Job drawing, mm, ordinate dimensions from the low corner. One solid piece. A direction names the side the tool comes from. Round coordinates to 2 decimals unless told otherwise and drop trailing zeros. Write each loop counter-clockwise with the first axis right and the second up, starting at its lowest first coordinate (ties: lowest second). Pieces come first, ordered by that corner, then holes.
1) Which spindle directions (+Z, -Z, +X, -X, +Y, -Y) get a long thin tool onto all of the face, cutting with end or side? Do the marked faces 1 and 2. Say none if no direction does.
2) Saw through at D-D (z = 9.75). Write the cut outline in (x, y).
3) Flat gauge pin, fed straight in: pin 1 (12 mm diameter, centred on x = 17.5, y = 18.5, fed in from +Z). Where does the tip first touch, or does it go through?
4) Saw through at A-A (y = 27.5). Write the cut outline in (x, z).
5) Saw through at B-B (x = 52.5). Write the cut outline in (y, z), plus the area to 3 significant figures.
6) Wall check: probe 1 along Y at (x, z) = (7.75, 6); probe 2 along Y at (x, z) = (2.5, 6); probe 3 along X at (y, z) = (19, 9). Give the ranges that are in metal, low to high.
7) Saw through at C-C (z = 6). Write the cut outline in (x, y).
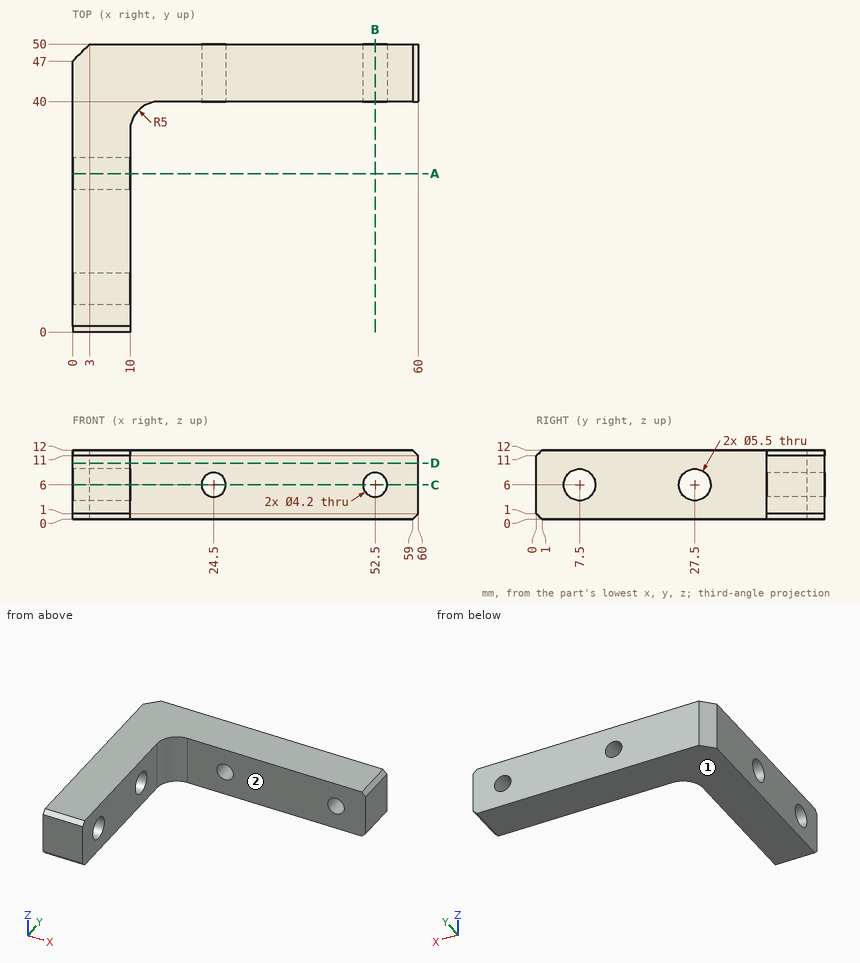
Evaluation:
1. face 1: -Z, +X, -X, +Y, -Y
1. face 2: +Z, -Z, +X, -Y
2. outline: (0, 0) - (10, 0) - (10, 35) arc R5 cw to (15, 40) - (60, 40) - (60, 50) - (3, 50) - (0, 47) - close
3. pin 1: passes through
4. outline: (0, 0) - (10, 0) - (10, 3.25) - (0, 3.25) - close; (0, 8.75) - (10, 8.75) - (10, 12) - (0, 12) - close
5. outline: (40, 0) - (50, 0) - (50, 3.9) - (40, 3.9) - close; (40, 8.1) - (50, 8.1) - (50, 12) - (40, 12) - close
5. area: 78.0 mm2
6. probe 1: y = 0 to 4.75, 10.25 to 24.75, 30.25 to 50
6. probe 2: y = 0 to 4.75, 10.25 to 24.75, 30.25 to 49.5
6. probe 3: x = 0 to 10
7. outline: (0, 0) - (10, 0) - (10, 4.75) - (0, 4.75) - close; (0, 10.25) - (10, 10.25) - (10, 24.75) - (0, 24.75) - close; (0, 30.25) - (10, 30.25) - (10, 35) arc R5 cw to (15, 40) - (22.4, 40) - (22.4, 50) - (3, 50) - (0, 47) - close; (26.6, 40) - (50.4, 40) - (50.4, 50) - (26.6, 50) - close; (54.6, 40) - (60, 40) - (60, 50) - (54.6, 50) - close
